from build123d import *

# Parameters (mm, degrees)
BLOCK_PROFILE_SKETCH_W         = 150
BLOCK_PROFILE_SKETCH_H         = 120
BASE_BLOCK_150X120X50_DEPTH    = 50
PORT_COUNTERBORE_SKETCH_R      = 22.55
PORT_COUNTERBORES_5_DEEP_DEPTH = 5
PORT_HOLE_SKETCH_R             = 17.5
PORT_HOLE_SKETCH_R_2           = 15.429011377
PORT_HOLE_SKETCH_R_3           = 15.274258873
PORT_HOLE_SKETCH_R_4           = 16.993106502
PORT_HOLE_SKETCH_R_5           = 15.982646342
PORT_HOLE_SKETCH_R_6           = 16.333623566
PORT_THROUGH_HOLES_DEPTH       = 198.294196569
EDGE_CHAMFER_10X45_A_SIZE      = 10
EDGE_CHAMFER_10X45_B_SIZE      = 10
MOUNTING_EARS_DEPTH            = 17
EAR_HOLE_SKETCH_R              = 5.5
EAR_HOLES_DEPTH                = 15
SIDE_RECESS_SKETCH_R           = 13
SIDE_RECESS_DEPTH              = 25


with BuildPart() as part:
    # Block Profile Sketch → Base Block 150x120x50 (new body)
    with BuildSketch(Plane.XY):
        with Locations((75, 60)):
            Rectangle(BLOCK_PROFILE_SKETCH_W, BLOCK_PROFILE_SKETCH_H)
    extrude(amount=BASE_BLOCK_150X120X50_DEPTH)

    # Port Counterbore Sketch → Port Counterbores 5 Deep (cut)
    with BuildSketch(Plane(origin=(0, 0, 0), x_dir=(-1, 0, 0), z_dir=(0, 0, -1))):
        with Locations((-125, 87.5)):
            Circle(PORT_COUNTERBORE_SKETCH_R)
        with Locations((-75, 87.5)):
            Circle(PORT_COUNTERBORE_SKETCH_R)
        with Locations((-25, 87.5)):
            Circle(PORT_COUNTERBORE_SKETCH_R)
        with Locations((-25, 32.5)):
            Circle(PORT_COUNTERBORE_SKETCH_R)
        with Locations((-75, 32.5)):
            Circle(PORT_COUNTERBORE_SKETCH_R)
        with Locations((-125, 32.5)):
            Circle(PORT_COUNTERBORE_SKETCH_R)
    extrude(amount=-PORT_COUNTERBORES_5_DEEP_DEPTH, mode=Mode.SUBTRACT)

    # Port Hole Sketch → Port Through Holes (cut, through all)
    with BuildSketch(Plane(origin=(0, 0, 5), x_dir=(-1, 0, 0), z_dir=(0, 0, -1))):
        with Locations((-125, 87.5)):
            Circle(PORT_HOLE_SKETCH_R)
        with Locations((-75, 87.5)):
            Circle(PORT_HOLE_SKETCH_R_2)
        with Locations((-25, 87.5)):
            Circle(PORT_HOLE_SKETCH_R_3)
        with Locations((-125, 32.5)):
            Circle(PORT_HOLE_SKETCH_R_4)
        with Locations((-75, 32.5)):
            Circle(PORT_HOLE_SKETCH_R_5)
        with Locations((-25, 32.5)):
            Circle(PORT_HOLE_SKETCH_R_6)
    extrude(amount=-PORT_THROUGH_HOLES_DEPTH, mode=Mode.SUBTRACT)

    # Edge Chamfer 10x45 A
    edge_chamfer_10x45_a_edges = [part.edges().sort_by_distance(p)[0] for p in [
        (0, 0, 25),
    ]]
    chamfer(edge_chamfer_10x45_a_edges, length=EDGE_CHAMFER_10X45_A_SIZE)

    # Edge Chamfer 10x45 B
    edge_chamfer_10x45_b_edges = [part.edges().sort_by_distance(p)[0] for p in [
        (0, 120, 25),
        (150, 120, 25),
        (150, 0, 25),
    ]]
    chamfer(edge_chamfer_10x45_b_edges, length=EDGE_CHAMFER_10X45_B_SIZE)

    # Mounting Ear Profile Sketch → Mounting Ears (add)
    with BuildSketch(Plane.XY.offset(50)):
        with BuildLine():
            Line((0, 79.364916731), (0, 40.635083269))
            ThreePointArc((0, 40.635083269), (-1.047152925, 43.696945447), (-3.75, 45.476312452))
            ThreePointArc((-3.75, 45.476312452), (-15, 60), (-3.75, 74.523687548))
            ThreePointArc((-3.75, 74.523687548), (-1.047152925, 76.303054553), (0, 79.364916731))
        make_face()
        with BuildLine():
            Line((150, 79.364916731), (150, 40.635083269))
            ThreePointArc((150, 40.635083269), (151.047152925, 43.696945447), (153.75, 45.476312452))
            ThreePointArc((153.75, 45.476312452), (165, 60), (153.75, 74.523687548))
            ThreePointArc((153.75, 74.523687548), (151.047152925, 76.303054553), (150, 79.364916731))
        make_face()
    extrude(amount=-MOUNTING_EARS_DEPTH)

    # Ear Hole Sketch → Ear Holes (cut)
    with BuildSketch(Plane.XY.offset(50)):
        with Locations((150, 60)):
            Circle(EAR_HOLE_SKETCH_R)
        with Locations((0, 60)):
            Circle(EAR_HOLE_SKETCH_R)
    extrude(amount=-EAR_HOLES_DEPTH, mode=Mode.SUBTRACT)

    # Side Recess Sketch → Side Recess (cut)
    with BuildSketch(Plane.XY.offset(50)):
        with Locations((47.5, 60)):
            Circle(SIDE_RECESS_SKETCH_R)
        with Locations((97.5, 60)):
            Circle(SIDE_RECESS_SKETCH_R)
    extrude(amount=-SIDE_RECESS_DEPTH, mode=Mode.SUBTRACT)


solid = part.part
The model under review builds one solid part; all positions refer to its coordinate system, in mm. A direction names the side the tool comes from. Coordinates: 2 decimals unless noted, no trailing zeros. Write each loop counter-clockwise with the first axis right and the second up, starting at its lowest first coordinate (ties: lowest second). Pieces come first, ordered by that corner, then holes. Notation, with made-up numbers: (6, 46.5) - (25, 46.5) arc R35 ccw to (25, 80.5) - close; hole circle Ø5 at (80.5, -1.75). An arc over 180 degrees is marked (long way). Answer as a JSON object with one key per item and string values. Group by question number.
1. Add section C-C (z = 17). Give the boundary of the cut face in (x, y).
2. To check wall thickness, follow probe 1 along Y at (x, z) = (75, 3.3); probe 2 along X at (y, z) = (32, 3); probe 3 along Y at (x, z) = (124, 9). State the ranges of each line that lie inside material, in increasing order.
3. Mouldability with a two-part tool opening along X and no side actions: class faces 5 (the face through (5, 5, 25)), 6 (the face through (113, 74, 5)), 7 (the face through (145, 5, 25)) as pulls with the +X half, pulls with the -X half, needs draft (parallel to the pull), parting line crosses it, or undercut.
4. Add section D-D (x = 25). Give the boundary of the cut face in (y, z).
5. Add section A-A (x = 75). Give the boundary of the cut face in (y, z).
6. Add section B-B (y = 97.5). Give the boundary of the cut face in (x, z), plus the area to 3 significant figures.
7. Machinability: for faces 1 (the face through (0, 59, 25)), 2 (the face through (-6, 60, 33)), 3 (the face through (41.62, 47.74, 2.46)), 4 (the face through (47, 60, 25)), which of the approach directions +Z, -Z, +X, -X, +Y, -Y give a long, thin tool a straight path to every point of the face, cutting with its end or side? Answer none if there is none.
8. Clearance check with flat-ended pins moving along their axes: pin 1 Ø13 at (x, y) = (42.5, 56.5) entering from +Z; pin 2 Ø5 at (y, z) = (53.5, 12.5) entering from +X; pin 3 Ø22.5 at (x, y) = (20, 27) entering from -Z. State where each tip first meets the part, or that it passes through.
Findings:
{
 "1": {"outline": "(0, 10) - (10, 0) - (140, 0) - (150, 10) - (150, 110) - (140, 120) - (10, 120) - (0, 110) - close; hole circle Ø32.67 at (25, 32.5); hole circle Ø30.55 at (25, 87.5); hole circle Ø31.97 at (75, 32.5); hole circle Ø30.86 at (75, 87.5); hole circle Ø35 at (125, 87.5); hole circle Ø33.99 at (125, 32.5)"},
 "2": {"probe 1": "0 to 9.95, 55.05 to 64.95, 110.05 to 120", "probe 2": "0 to 2.46, 47.54 to 52.46, 97.54 to 102.46, 147.54 to 150", "probe 3": "0 to 15.54, 49.46 to 70.03, 104.97 to 120"},
 "3": {"face 5": "pulls with the -X half", "face 6": "undercut", "face 7": "pulls with the +X half"},
 "4": {"outline": "(0, 0) - (9.95, 0) - (9.95, 5) - (16.17, 5) - (16.17, 50) - (0, 50) - close; (48.83, 5) - (55.05, 5) - (55.05, 0) - (64.95, 0) - (64.95, 5) - (72.23, 5) - (72.23, 50) - (48.83, 50) - close; (102.77, 5) - (110.05, 5) - (110.05, 0) - (120, 0) - (120, 50) - (102.77, 50) - close"},
 "5": {"outline": "(0, 0) - (9.95, 0) - (9.95, 5) - (16.52, 5) - (16.52, 50) - (0, 50) - close; (48.48, 5) - (55.05, 5) - (55.05, 0) - (64.95, 0) - (64.95, 5) - (72.07, 5) - (72.07, 50) - (48.48, 50) - close; (102.93, 5) - (110.05, 5) - (110.05, 0) - (120, 0) - (120, 50) - (102.93, 50) - close"},
 "6": {"outline": "(0, 0) - (4.79, 0) - (4.79, 5) - (13.45, 5) - (13.45, 50) - (0, 50) - close; (36.55, 5) - (45.21, 5) - (45.21, 0) - (54.79, 0) - (54.79, 5) - (63.25, 5) - (63.25, 50) - (36.55, 50) - close; (86.75, 5) - (95.21, 5) - (95.21, 0) - (104.79, 0) - (104.79, 5) - (110.64, 5) - (110.64, 50) - (86.75, 50) - close; (139.36, 5) - (145.21, 5) - (145.21, 0) - (150, 0) - (150, 50) - (139.36, 50) - close", "area": "3,500 mm²"},
 "7": {"face 1": "-Z, -X", "face 2": "-Z, -X, +Y, -Y", "face 3": "-Z", "face 4": "+Z"},
 "8": {"pin 1": "z = 25", "pin 2": "x = 150", "pin 3": "z = 5"}
}
